from build123d import *

# Parameters (mm, degrees)
SKETCH1_W           = 300
SKETCH1_H           = 200
BOSS_EXTRUDE1_DEPTH = 30
SKETCH2_R           = 15
SKETCH2_R_2         = 5
CUT_EXTRUDE1_DEPTH  = 30
FILLET1_R           = 30


with BuildPart() as part:
    # Sketch1 → Boss-Extrude1 (new body)
    with BuildSketch(Plane(origin=(0, 0, 0), x_dir=(1, 0, 0), z_dir=(0, 1, 0))):
        Rectangle(SKETCH1_W, SKETCH1_H)
    extrude(amount=BOSS_EXTRUDE1_DEPTH)

    # Sketch2 → Cut-Extrude1 (cut)
    with BuildSketch(Plane(origin=(0, 30, 0), x_dir=(1, 0, 0), z_dir=(0, 1, 0))):
        with Locations(Location((0, 0, 0), (0, 0, 270))):
            Circle(SKETCH2_R)
        with Locations(Location((0, 45, 0), (0, 0, 270))):
            Circle(SKETCH2_R_2)
        with Locations(Location((-45, 0, 0), (0, 0, 270))):
            Circle(SKETCH2_R_2)
        with Locations(Location((0, -45, 0), (0, 0, 90))):
            Circle(SKETCH2_R_2)
        with Locations(Location((45, 0, 0), (0, 0, 90))):
            Circle(SKETCH2_R_2)
    extrude(amount=-CUT_EXTRUDE1_DEPTH, mode=Mode.SUBTRACT)

    # Fillet1
    fillet1_edges = [part.edges().sort_by_distance(p)[0] for p in [
        (150, 15, 100),
        (-150, 15, 100),
        (-150, 15, -100),
        (150, 15, -100),
    ]]
    fillet(fillet1_edges, radius=FILLET1_R)


solid = part.part
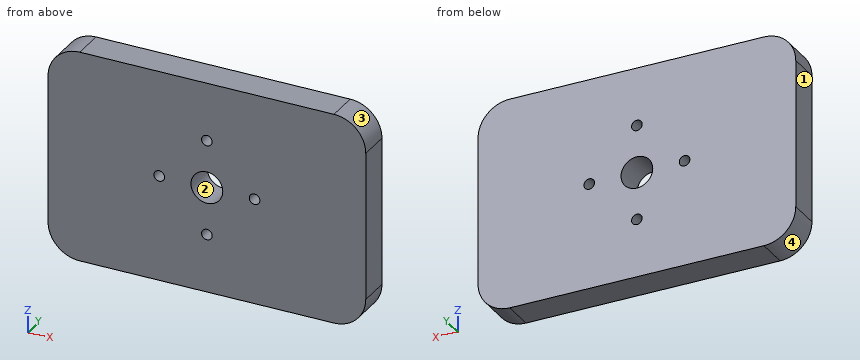
The listing builds one solid part. Answer for the finished solid, in the listing's coordinates (mm). Face numbers are marked on the shaded views. Round coordinates to 2 decimals unless told otherwise and drop trailing zeros. Loops run counter-clockwise (first coordinate to the right, second up) from the corner with the lowest first, then second, coordinate; pieces in that order, holes last. Notation, with made-up numbers: M -9,-27 L 47,-27 A25 cw 47,9 Z; hole C 51,20 d11. An arc over 180 degrees is marked long. Write each question's results on one line, items separated by ' | '. Start each with the question number.
1) Determine the mould class of the marked faces 1, 2, 3 and 4 for opening direction Z: pulls with the +Z half, pulls with the -Z half, needs draft (parallel to the pull), parting line crosses it, or undercut.
2) Find section D-D on x = 0. Write down the section's boundary in (y, z), plus the area to 3 significant figures.
3) Find section A-A on x = -45. Write down the section's boundary in (y, z).
4) Find section C-C on y = 25. Write down the section's boundary in (x, z).
5) This flat-tipped pin is pushed along its axis until it touches: pin 1 (18 mm diameter, centred on x = 0, z = 0, fed in from -Y). Where does it stop, or does it pass through?
6) Find section B-B on z = -45. Write down the section's boundary in (x, y), plus the area to 3 significant figures.
7) Straight lines are drawn through the part: probe 1 along X at (y, z) = (7.75, 0); probe 2 along Z at (x, y) = (45, 22.25); probe 3 along X at (y, z) = (15, 3.5). For each, find the intervals that lie inside material, in ascending order.
Final values:
1) face 1: needs draft | face 2: undercut | face 3: pulls with the +Z half | face 4: pulls with the -Z half
2) outline: M 0,-100 L 30,-100 L 30,-50 L 0,-50 Z; M 0,-40 L 30,-40 L 30,-15 L 0,-15 Z; M 0,15 L 30,15 L 30,40 L 0,40 Z; M 0,50 L 30,50 L 30,100 L 0,100 Z | area: 4,500 mm²
3) outline: M 0,-100 L 30,-100 L 30,-5 L 0,-5 Z; M 0,5 L 30,5 L 30,100 L 0,100 Z
4) outline: M -150,-70 A30 ccw -120,-100 L 120,-100 A30 ccw 150,-70 L 150,70 A30 ccw 120,100 L -120,100 A30 ccw -150,70 Z; hole C -45,0 d10; hole C 0,0 d30; hole C 0,-45 d10; hole C 0,45 d10; hole C 45,0 d10
5) pin 1: through
6) outline: M -150,0 L -5,0 L -5,30 L -150,30 Z; M 5,0 L 150,0 L 150,30 L 5,30 Z | area: 8,700 mm²
7) probe 1: -150 to -50, -40 to -15, 15 to 40, 50 to 150 | probe 2: -100 to -5, 5 to 100 | probe 3: -150 to -48.57, -41.43 to -14.59, 14.59 to 41.43, 48.57 to 150
